from build123d import *

# Parameters (mm, degrees)
SKETCH_1_W                = 120
SKETCH_1_H                = 100
EXTRUDE_1_DEPTH           = 20
HOLE_WIZARD_1_D           = 9
HOLE_WIZARD_1_CBORE_D     = 15
HOLE_WIZARD_1_CBORE_DEPTH = 9
SKETCH_4_R                = 15
CUT_EXTRUDE_1_DEPTH       = 81.622577483
HOLE_WIZARD_M8_1_D        = 6.8


with BuildPart() as part:
    # 草图1 → 凸台-拉伸1 (new body)
    with BuildSketch(Plane(origin=(0, 0, 0), x_dir=(0, 0, -1), z_dir=(1, 0, 0))):
        Rectangle(SKETCH_1_W, SKETCH_1_H)
    extrude(amount=EXTRUDE_1_DEPTH)

    # 打孔尺寸(%根据)内六角圆柱头螺钉的类型1 (through all)
    with Locations(Plane(origin=(20, 0, 0), x_dir=(0, 0, -1), z_dir=(1, 0, 0))):
        with Locations((-35, 30), (15, 30), (-35, -30), (15, -30)):
            CounterBoreHole(HOLE_WIZARD_1_D / 2, HOLE_WIZARD_1_CBORE_D / 2, HOLE_WIZARD_1_CBORE_DEPTH)

    # 草图4 → 切除-拉伸1 (cut, through all)
    with BuildSketch(Plane(origin=(20, 0, 0), x_dir=(0, 0, -1), z_dir=(1, 0, 0))):
        with Locations((-10, 0)):
            Circle(SKETCH_4_R)
    extrude(amount=-CUT_EXTRUDE_1_DEPTH, mode=Mode.SUBTRACT)

    # M8 螺纹孔1 (through all)
    with Locations(Plane(origin=(20, 0, 0), x_dir=(0, 0, -1), z_dir=(1, 0, 0))):
        with Locations((-50, 40), (-50, -40), (50, -40), (50, 40)):
            Hole(HOLE_WIZARD_M8_1_D / 2)


solid = part.part
Could you check a few things on this model? Use its own coordinates, in mm. A direction names the side the tool comes from. Round coordinates to 2 decimals unless told otherwise and drop trailing zeros. Order: outer loops, then holes, each group sorted by start corner. A loop starts at its lowest first (then second) coordinate and runs counter-clockwise, first axis right, second up.
(1) Imagine slicing it at A-A (y = 30). Write out the boundary of the cut face in (x, z), plus the area to 3 significant figures.
Response values:
outline: (0, -60) - (20, -60) - (20, -22.5) - (11, -22.5) - (11, -19.5) - (0, -19.5) - close; (0, -10.5) - (11, -10.5) - (11, -7.5) - (20, -7.5) - (20, 27.5) - (11, 27.5) - (11, 30.5) - (0, 30.5) - close; (0, 39.5) - (11, 39.5) - (11, 42.5) - (20, 42.5) - (20, 60) - (0, 60) - close
area: 1,930 mm2
(2) Imagine slicing it at D-D (z = 10). Write out the boundary of the cut face in (x, y), plus the area to 3 significant figures.
Response values:
outline: (0, -50) - (20, -50) - (20, -15) - (0, -15) - close; (0, 15) - (20, 15) - (20, 50) - (0, 50) - close
area: 1,400 mm2
(3) Imagine slicing it at B-B (z = -15). Write out the boundary of the cut face in (x, y), plus the area to 3 significant figures.
Response values:
outline: (0, -50) - (20, -50) - (20, -37.5) - (11, -37.5) - (11, -34.5) - (0, -34.5) - close; (0, -25.5) - (11, -25.5) - (11, -22.5) - (20, -22.5) - (20, 22.5) - (11, 22.5) - (11, 25.5) - (0, 25.5) - close; (0, 34.5) - (11, 34.5) - (11, 37.5) - (20, 37.5) - (20, 50) - (0, 50) - close
area: 1,530 mm2
(4) If we mould it in two halves opening along Y, with no side actions, what happens to faces 3 (the flat face through (11, 30, -20)), 4 (the flat face through (10, -50, 1)), 5 (the flat face through (0, 1, -12)), 6 (the flat face through (11, 30, 30))? For each: released by +Y, released by -Y, zero draft, split by the parting line, or undercut.
Response values:
face 3: undercut
face 4: released by -Y
face 5: zero draft
face 6: undercut
(5) Please list where these lines run through material, in increasing order: line 1 along Y through (x, z) = (16.25, 35); line 2 along Y through (x, z) = (8.5, 35); line 3 along Z through (x, y) = (2.75, -33).
Response values:
line 1: y = -50 to -37.5, -22.5 to 22.5, 37.5 to 50
line 2: y = -50 to -34.5, -25.5 to 25.5, 34.5 to 50
line 3: z = -60 to -18.35, -11.65 to 31.65, 38.35 to 60
(6) Imagine slicing it at C-C (x = 5.5). Count the separate pieces of the cut face and the enclosed holes in it, plus the area to 3 significant figures.
Response values:
separate pieces: 1
enclosed holes: 9
area: 10,900 mm2
(7) Which directions (+Z, -Z, +X, -X, +Y, -Y) give clear straight access to the entire face, cutting with the end or side of a thin tool? Please do faces 1 (the flat face through (10, -1, -60)), 2 (the cylindrical face through (15.56, -37.32, 36.63)).
Response values:
face 1: -Z, +X, -X, +Y, -Y
face 2: +X
(8) I'm going to push a flat-ended pin straight in: pin 1 (4.5 mm diameter, centred on y = -27, z = 38.5, fed in from +X). Where does the tip first touch, or does it pass through?
Response values:
pin 1: stops at x = 11
